```python
from build123d import *

# Parameters (mm, degrees)
SKETCH_1_R      = 6
EXTRUDE_1_DEPTH = 12
SKETCH_2_R      = 3
EXTRUDE_2_DEPTH = 25
FILLET_1_R      = 1


with BuildPart() as part:
    # 草图1 → 凸台-拉伸1 (new body)
    with BuildSketch(Plane(origin=(0, 0, 0), x_dir=(1, 0, 0), z_dir=(0, 1, 0))):
        with Locations(Location((0, 0, 0), (0, 0, 270))):
            Circle(SKETCH_1_R)
    extrude(amount=EXTRUDE_1_DEPTH)

    # 草图2 → 凸台-拉伸2 (add)
    with BuildSketch(Plane(origin=(0, 12, 0), x_dir=(1, 0, 0), z_dir=(0, 1, 0))):
        with Locations(Location((0, 0, 0), (0, 0, 270))):
            Circle(SKETCH_2_R)
    extrude(amount=EXTRUDE_2_DEPTH)

    # 圆角1
    fillet_1_edges = [part.edges().sort_by_distance(p)[0] for p in [
        (0, 0, -6),
        (0, 12, -6),
        (0, 37, -3),
    ]]
    fillet(fillet_1_edges, radius=FILLET_1_R)


solid = part.part
```
Design review of the part built by this model. Coordinates are the model's own, in mm. A direction names the side the tool comes from. Coordinates: 2 decimals unless noted, no trailing zeros. Order: outer loops, then holes, each group sorted by start corner. A loop starts at its lowest first (then second) coordinate and runs counter-clockwise, first axis right, second up. Notation, with made-up numbers: (20, 44) - (74, 44) arc R19 cw to (74, 57) - close; hole circle Ø3 at (32, 51.5). An arc over 180 degrees is marked (long way). One line per question, with ' | ' between items.
Q1. Clearance check with flat-ended pins moving along their axes: pin 1 Ø2 at (x, y) = (-3, 5.5) entering from -Z; pin 2 Ø4 at (y, z) = (27, 3) entering from -X; pin 3 Ø4 at (x, y) = (3, 13.5) entering from -Z; pin 4 Ø1.5 at (x, z) = (4.5, 1) entering from -Y. State where each tip first meets the part, or that it passes through.
Answer key:
pin 1: stops at z = -5.66 | pin 2: stops at x = -2.83 | pin 3: stops at z = -5.31 | pin 4: stops at y = 0
Q2. To check wall thickness, follow line 1 along Y through (x, z) = (-2.75, -4.25); line 2 along Z through (x, y) = (-1.5, 35.5); line 3 along X through (y, z) = (27, 1.75). State the ranges of each line that lie inside material, in increasing order.
Answer key:
line 1: y = 0 to 12 | line 2: z = -2.6 to 2.6 | line 3: x = -2.44 to 2.44
Q3. Consider section B-B, the plane x = 0. Give the boundary of the cut face in (y, z).
Answer key:
outline: (0, -5) arc R1 ccw to (1, -6) - (11, -6) arc R1 ccw to (12, -5) - (12, -3) - (36, -3) arc R1 ccw to (37, -2) - (37, 2) arc R1 ccw to (36, 3) - (12, 3) - (12, 5) arc R1 ccw to (11, 6) - (1, 6) arc R1 ccw to (0, 5) - close
Q4. Consider section C-C, the plane y = 4.5. Give the boundary of the cut face in (x, z), then the cut area to 3 significant figures.
Answer key:
outline: circle Ø12 at (0, 0) | area: 113 mm2
Q5. For faces 1 (the flat face through (-3.3, 12, -0.1)), 2 (the flat face through (0, 37, 0)), list the 3-axis set-ups (+Z, -Z, +X, -X, +Y, -Y) from which the entire face can be reached by the end or side of a thin tool; tool diameter is ignored.
Answer key:
face 1: +Y | face 2: +Z, -Z, +X, -X, +Y
Q6. Consider section A-A, the plane z = 0. Give the boundary of the cut face in (x, y), then the cut area to 3 significant figures.
Answer key:
outline: (-6, 1) arc R1 ccw to (-5, 0) - (5, 0) arc R1 ccw to (6, 1) - (6, 11) arc R1 ccw to (5, 12) - (3, 12) - (3, 36) arc R1 ccw to (2, 37) - (-2, 37) arc R1 ccw to (-3, 36) - (-3, 12) - (-5, 12) arc R1 ccw to (-6, 11) - close | area: 293 mm2
Q7. Consider section D-D, the plane y = 34. Give the boundary of the cut face in (x, z).
Answer key:
outline: circle Ø6 at (0, 0)
